Verification items for the finished model (mm, model axes). A direction names the side the tool comes from. Give positions to 0.01 mm unless a question says otherwise; leave off trailing zeros. Write each loop counter-clockwise with the first axis right and the second up, starting at its lowest first coordinate (ties: lowest second). Pieces come first, ordered by that corner, then holes.
from build123d import *

# Parameters (mm, degrees)
BOSS_EXTRUDE1_DEPTH = 10
SKETCH4_R           = 26.75
SKETCH4_R_2         = 12
CUT_EXTRUDE1_DEPTH  = 1.25
CUT_EXTRUDE1_DRAFT  = -60
CHAMFER2_SIZE       = 0.888888889


with BuildPart() as part:
    # Sketch3 → Boss-Extrude1 (new body)
    with BuildSketch(Plane(origin=(0, 0, 0), x_dir=(0, 0, -1), z_dir=(1, 0, 0))):
        Polygon((12, 6.92820323), (0, 13.856406461), (-12, 6.92820323), (-12, -6.92820323), (0, -13.856406461), (12, -6.92820323), align=None)
    extrude(amount=BOSS_EXTRUDE1_DEPTH)


with BuildPart() as cut_extrude1_tool:
    # Sketch4 → Cut-Extrude1 (with draft: the straight prism first)
    with BuildSketch(Plane.ZY):
        Circle(SKETCH4_R)
        Circle(SKETCH4_R_2, mode=Mode.SUBTRACT)
    extrude(amount=-CUT_EXTRUDE1_DEPTH)
    # Cut-Extrude1: the draft: its side faces are tilted about the plane it starts from
    cut_extrude1_sides = [cut_extrude1_tool.faces().sort_by_distance(p)[0] for p in [
        (0.625, 0, -26.75),
        (0.625, 0, -12),
    ]]
    draft(cut_extrude1_sides, Plane.ZY, CUT_EXTRUDE1_DRAFT)


with BuildPart() as part_1:
    add(part.part)

    # Cut-Extrude1: cut by cut_extrude1_tool
    add(cut_extrude1_tool.part, mode=Mode.SUBTRACT)

    # Sketch5 → Revolve1 (revolve)
    with BuildSketch(Plane.XY, mode=Mode.PRIVATE) as revolve1_sk:
        with BuildLine():
            Line((10.85, 8), (130, 8))
            Line((130, 8), (130, 0))
            Line((130, 0), (10, 0))
            Line((10, 0), (10, 8.85))
            ThreePointArc((10, 8.85), (10.248959236, 8.248959236), (10.85, 8))
        make_face()
    revolve(revolve1_sk.sketch.rotate(Axis((10, 0, 0), (1, 0, 0)), 90), axis=Axis((10, 0, 0), (1, 0, 0)))

    # Chamfer2
    chamfer2_edges = [part_1.edges().sort_by_distance(p)[0] for p in [
        (130, 0, -8),
    ]]
    chamfer(chamfer2_edges, length=CHAMFER2_SIZE)

    # Sketch7 → Cut-Revolve1 (revolve, cut)
    with BuildSketch(Plane.XY, mode=Mode.PRIVATE) as cut_revolve1_sk:
        Polygon((10, 11.145), (9.2, 11.945), (9.2, 26.75), (10, 26.75), align=None)
    revolve(cut_revolve1_sk.sketch.rotate(Axis((0, 0, 0), (1, 0, 0)), 90), axis=Axis((0, 0, 0), (1, 0, 0)), mode=Mode.SUBTRACT)


solid = part_1.part
Item 1: Scan lines: line 1 along X through (y, z) = (-2.5, 9.75); line 2 along Y through (x, z) = (53, -4.5); line 3 along Y through (x, z) = (91.5, 1.75). Record each from-to range of solid material in increasing order.
Answer key:
line 1: x = 0 to 10
line 2: y = -6.61 to 6.61
line 3: y = -7.81 to 7.81
Item 2: Sectioned sample at A-A on x = 109. Record the cut outline in (y, z), then the cut area to 3 significant figures.
Answer key:
outline: circle Ø16 at (0, 0)
area: 201 mm2
Item 3: Release check for a two-part mould opening along Z. For faces 1 (the face through (0.256, -12.443, -0.03)), 2 (the face through (4.54, 10.44, 5.92)), 3 (the face through (5, 0, -12)), 4 (the face through (130, 0, 0)) record: released by +Z, released by -Z, zero draft, split by the parting line, or undercut.
Answer key:
face 1: split by the parting line
face 2: released by +Z
face 3: released by -Z
face 4: zero draft
Item 4: Set-up check for faces 5 (the face through (9.2, 12.3, 0.9)), 6 (the face through (0.256, -6.195, -10.791)): record each of +Z, -Z, +X, -X, +Y, -Y from which the full face is reachable in a straight line by a thin tool's end or side.
Answer key:
face 5: +X
face 6: -Z, -X, -Y
Item 5: Depth check by flat-ended pin: pin 1 (12 mm diameter, centred on x = 51, z = 6.5, fed in from +Y); pin 2 (6 mm diameter, centred on x = 63, y = -10, fed in from +Z); pin 3 (10 mm diameter, centred on x = 83.5, z = 1.5, fed in from -Y); pin 4 (1 mm diameter, centred on x = 112.5, y = -10, fed in from +Z). Enter the tip coordinate at first touch or a pass-through.
Answer key:
pin 1: stops at y = 7.98
pin 2: stops at z = 3.87
pin 3: stops at y = -8
pin 4: passes through
